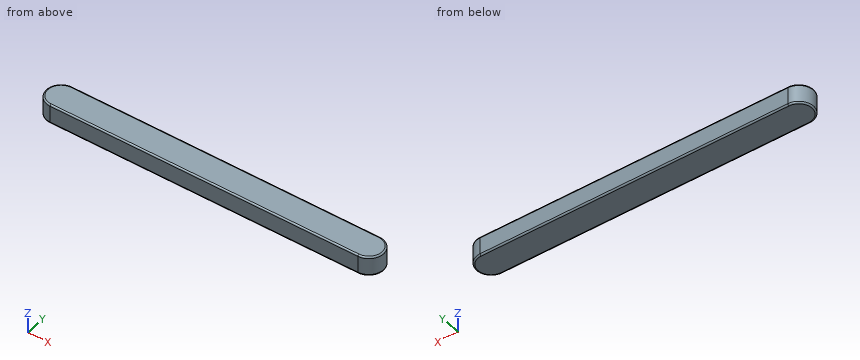
from build123d import *

# Parameters (mm, degrees)
EXTRUDE_523_DEPTH = 8
FILLET_1_R        = 0.6


with BuildPart() as part:
    # 草图1 → Extrude 523 (new body)
    with BuildSketch(Plane.XY):
        with BuildLine():
            Line((-64, 6), (64, 6))
            ThreePointArc((64, 6), (70, 0), (64, -6))
            Line((64, -6), (-64, -6))
            ThreePointArc((-64, -6), (-70, 0), (-64, 6))
        make_face()
    extrude(amount=EXTRUDE_523_DEPTH)

    # 圆角1
    fillet_1_edges = [part.edges().sort_by_distance(p)[0] for p in [
        (70, 0, 8),
        (0, 6, 8),
        (-70, 0, 8),
        (0, 6, 0),
        (70, 0, 0),
        (0, -6, 0),
        (-70, 0, 0),
        (0, -6, 8),
    ]]
    fillet(fillet_1_edges, radius=FILLET_1_R)


solid = part.part
Source: CAD feature listing. Evaluate the final solid. Frame: model axes, mm. Coordinates: 2 decimals unless noted, no trailing zeros. Order: outer loops, then holes, each group sorted by start corner. A loop starts at its lowest first (then second) coordinate and runs counter-clockwise, first axis right, second up. Notation, with made-up numbers: M 42.25,58 L 46.25,58 A13 ccw 46.25,72 Z; hole C 63,-14 d7. An arc over 180 degrees is marked long. Write each question's results on one line, items separated by ' | '. Start each with the question number.
Item 1: Cut plane A-A (z = 6.25). Return loops of the section in (x, y).
Item 2: Line query: probe 1 along Y at (x, z) = (48.5, 0.5); probe 2 along X at (y, z) = (1, 3.75); probe 3 along X at (y, z) = (2.25, 7.25). Output: solid intervals per line, ascending.
Item 3: First-contact query: pin 1 Ø1.5 at (y, z) = (2, 5.5) entering from -X. Flat tip, straight axial feed; report the tip coordinate or a pass-through.
Checked values:
1) outline: M -64,-6 L 64,-6 A6 ccw 64,6 L -64,6 A6 ccw Z
2) probe 1: y = -5.99 to 5.99 | probe 2: x = -69.92 to 69.92 | probe 3: x = -69.56 to 69.56
3) pin 1: stops at x = -69.87
